Design review of the part shown in the three views and the two pictorial views. Dimensions are in mm from the part's minimum x, y and z. Give positions to 0.01 mm unless a question says otherwise; leave off trailing zeros. Order: outer loops, then holes, each group sorted by start corner. A loop starts at its lowest first (then second) coordinate and runs counter-clockwise, first axis right, second up. Notation, with made-up numbers: (38.25, 62) -> (59.25, 62) arc R24 cw to (59.25, 100) -> close; hole circle Ø3 at (76, -17.75). An arc over 180 degrees is marked (long way). Use one line per item in the form item = value.
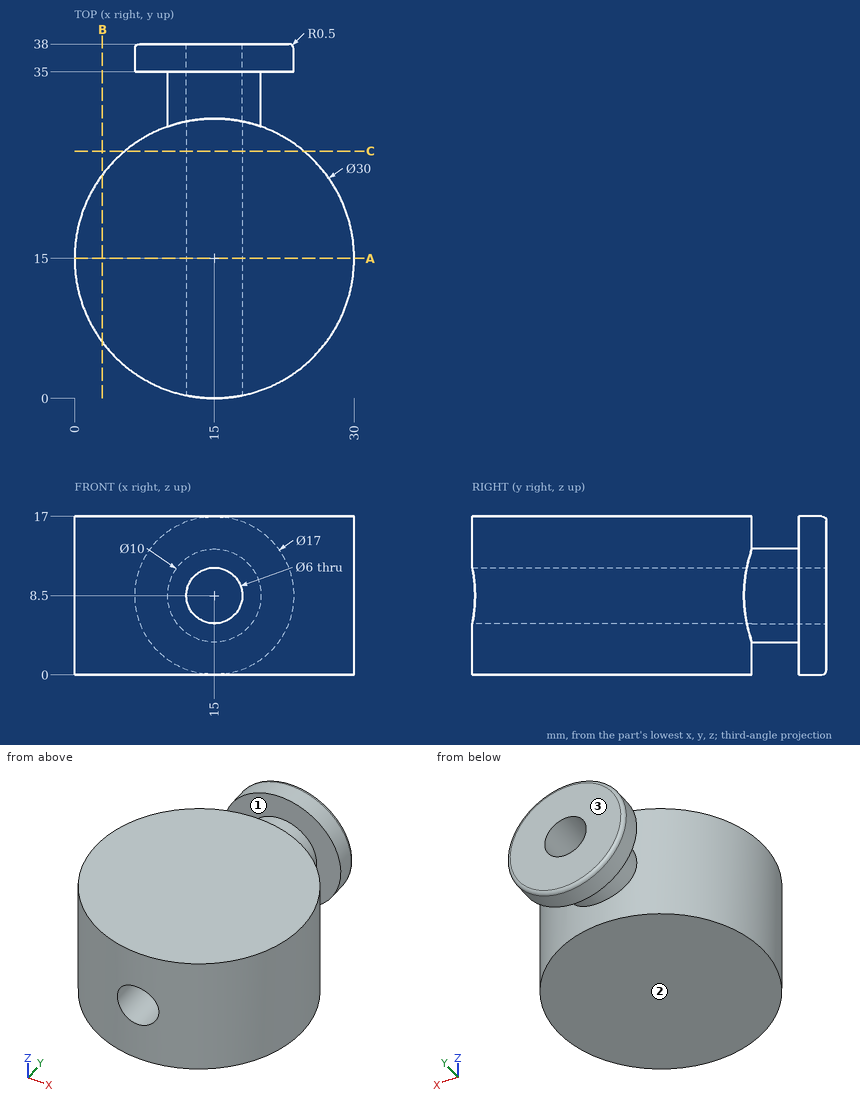
1. Add section A-A on y = 15. Give the boundary of the cut face in (x, z), then the cut area to 3 significant figures.
Values:
outline = (0, 0) -> (30, 0) -> (30, 17) -> (0, 17) -> close; hole circle Ø6 at (15, 8.5)
area = 482 mm^2
2. The part is to be moulded in two halves that separate along Y. For the marked faces 1, 2 and 3, say which applies: +Y half, -Y half, draft (parallel to the pull), parting line (faces both ways), or undercut.
Values:
face_1 = undercut
face_2 = draft
face_3 = +Y half
3. Add section C-C on y = 26.5. Give the boundary of the cut face in (x, z), then the cut area to 3 significant figures.
Values:
outline = (5.37, 0) -> (24.63, 0) -> (24.63, 17) -> (5.37, 17) -> close; hole circle Ø6 at (15, 8.5)
area = 299 mm^2
4. Add section B-B on x = 3. Give the boundary of the cut face in (y, z).
Values:
outline = (6, 0) -> (24, 0) -> (24, 17) -> (6, 17) -> close
5. For pin 1 Ø6 at (x, z) = (5.5, 3) entering from -Y; pin 2 Ø5 at (x, z) = (19.5, 11) entering from -Y; pin 3 Ø4 at (y, z) = (7.5, 4) entering from -X, all flat-tipped, find the tip position at first contact; note any pin that passes through.
Values:
pin_1 = 1.48
pin_2 = 0.13
pin_3 = 1.04
6. For L1, parallel to X at y = 35.75, z = 8.5; L2, parallel to X at y = 14, z = 8.5; L3, parallel to Z at x = 16, y = 34, list the stretches that pass through material, from the lowest coordinate up.
Values:
L1 = 6.5 to 12, 18 to 23.5
L2 = 0.03 to 12, 18 to 29.97
L3 = 3.6 to 5.67, 11.33 to 13.4
